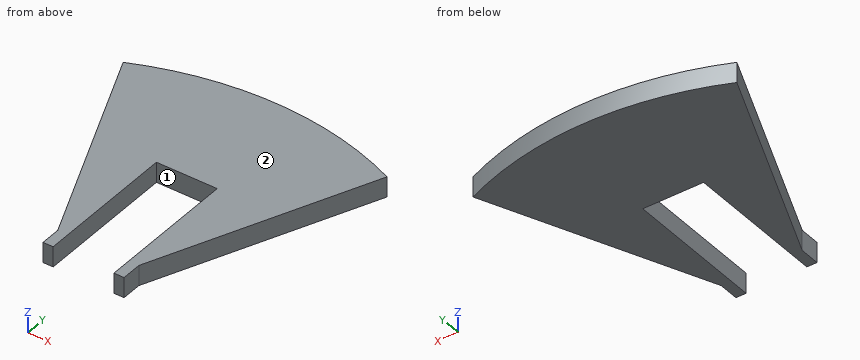
from build123d import *

# Parameters (mm, degrees)
BOSS_EXTRUDE2_DEPTH = 5


with BuildPart() as part:
    # Sketch1 → Boss-Extrude2 (new, symmetric)
    with BuildSketch(Plane.XY):
        with BuildLine():
            ThreePointArc((65.10089705, 147.251055016), (0, 161), (-65.10089705, 147.251055016))
            Line((-65.10089705, 147.251055016), (-20, 41))
            Line((-20, 41), (-20, 31))
            Line((-20, 31), (-15, 31))
            Line((-15, 31), (-15, 101))
            Line((-15, 101), (15, 101))
            Line((15, 101), (15, 31))
            Line((15, 31), (20, 31))
            Line((20, 31), (20, 41))
            Line((20, 41), (65.10089705, 147.251055016))
        make_face()
    extrude(amount=BOSS_EXTRUDE2_DEPTH, both=True)


solid = part.part
Geometry: final body of the model. Coordinates: model frame, mm. Face numbers are marked on the shaded views. A direction names the side the tool comes from. Give positions to 0.01 mm unless a question says otherwise; leave off trailing zeros. Loops run counter-clockwise (first coordinate to the right, second up) from the corner with the lowest first, then second, coordinate; pieces in that order, holes last. Notation, with made-up numbers: (-5.5, -4) -> (33.5, -4) arc R18 ccw to (33.5, 19) -> close; hole circle Ø5 at (38, 52). An arc over 180 degrees is marked (long way). Put each result on its own line as item: value.
1. Cut plane A-A (y = 58.5). Return the cut outline in (x, z).
Taken from the geometry:
outline: (-27.43, -5) -> (-15, -5) -> (-15, 5) -> (-27.43, 5) -> close; (15, -5) -> (27.43, -5) -> (27.43, 5) -> (15, 5) -> close
2. Pin query (flat end, axial travel): P1, Ø4, axis at y = 50, z = -3.5, coming from the -X side; P2, Ø5, axis at y = 79.5, z = 1, coming from the -X side; P3, Ø1, axis at y = 117.5, z = 0.5, coming from the +X side. Return the tip coordinate at first contact, or that it passes through.
Taken from the geometry:
P1: stops at x = -24.67
P2: stops at x = -37.4
P3: stops at x = 52.68
3. Ray query, line 1 along X through (y, z) = (40.5, 2); line 2 along X through (y, z) = (78, 4.5); line 3 along Y through (x, z) = (-1, 4). Return the intervals inside material, ascending. Write a range as [from, to].
Taken from the geometry:
line 1: x = [-20, -15], [15, 20]
line 2: x = [-35.71, -15], [15, 35.71]
line 3: y = [101, 161]
4. Cut plane C-C (y = 43.5). Return the cut outline in (x, z).
Taken from the geometry:
outline: (-21.06, -5) -> (-15, -5) -> (-15, 5) -> (-21.06, 5) -> close; (15, -5) -> (21.06, -5) -> (21.06, 5) -> (15, 5) -> close
5. Cut plane B-B (z = -1.5). Return the cut outline in (x, y).
Taken from the geometry:
outline: (-65.1, 147.25) -> (-20, 41) -> (-20, 31) -> (-15, 31) -> (-15, 101) -> (15, 101) -> (15, 31) -> (20, 31) -> (20, 41) -> (65.1, 147.25) arc R161 ccw to start
6. Set-up query: the marked faces 1 and 2. Return all of +Z, -Z, +X, -X, +Y, -Y with unobstructed straight access to the full face (end or side cutting, diameter ignored); none if empty.
Taken from the geometry:
face 1: +Z, -Z, -Y
face 2: +Z, +X, -X, +Y, -Y
7. Cut plane D-D (x = -2). Return the cut outline in (y, z).
Taken from the geometry:
outline: (101, -5) -> (160.99, -5) -> (160.99, 5) -> (101, 5) -> close
